Geometry check sheet. Reference: the model listing, model coordinates, mm. A direction names the side the tool comes from. Coordinates: 2 decimals unless noted, no trailing zeros. Write each loop counter-clockwise with the first axis right and the second up, starting at its lowest first coordinate (ties: lowest second). Pieces come first, ordered by that corner, then holes. Notation, with made-up numbers: (43.5, 63.5) -> (55.5, 63.5) arc R21 ccw to (55.5, 89.5) -> close; hole circle Ø4 at (-13.75, -30). An arc over 180 degrees is marked (long way). Answer in a Markdown table with one row per item. Add a question column.
1. Set-up check for faces 1 (the flat face through (12, 30, -48)), 2 (the flat face through (0, 9, 9)), 3 (the cylindrical face through (13.5, 4.4, 3.9)), 4 (the flat face through (0, 47, -52)), 5 (the flat face through (-4, 43, -30)): record each of +Z, -Z, +X, -X, +Y, -Y from which the full face is reachable in a straight line by a thin tool's end or side.
2. Scan lines: L1, parallel to Z at x = -10, y = 32; L2, parallel to Y at x = -5.75, z = -40; L3, parallel to Z at x = 18, y = 36. Record each from-to range of solid material in increasing order. Write a range as from..to.
3. Depth check by flat-ended pin: P1, Ø19, axis at y = 38.5, z = -33.5, coming from the +X side; P2, Ø5, axis at x = -7.5, y = 29, coming from the +Z side; P3, Ø6.5, axis at x = -16, y = 40, coming from the -Z side. Enter the tip coordinate at first touch or a pass-through.
4. Mould release check, pull along Z, two halves, no side actions. Record for faces 6 (the flat face through (0, 44, -8)), 7 (the cylindrical face through (0.056, 65.632, -54.374)), 8 (the cylindrical face through (17.352, 73.563, -35.708)), 9 (the cylindrical face through (-14.648, 73.563, -35.708)): pulls with the +Z half, pulls with the -Z half, needs draft (parallel to the pull), parting line crosses it, or undercut.
5. Cross-section at D-D on y = 72. Record the cut outline in (x, z), and give its area (3 significant figures).
6. Cross-section at C-C on y = 52. Record the cut outline in (x, z).
7. Cross-section at B-B on z = 1.5. Record the cut outline in (x, y).
8. Cross-section at A-A on x = -5. Record the cut outline in (y, z), and give its area (3 significant figures).
```python
from build123d import *
from build123d.topology import SkipClean

# Parameters (mm, degrees)
BASE_FOOT_WITH_SLOT_DEPTH     = 9
UPRIGHT_WALL_SKETCH_W         = 50
UPRIGHT_WALL_SKETCH_H         = 69
UPRIGHT_WALL_DEPTH            = 12
TOP_FLANGE_SKETCH_R           = 4.5
TOP_FLANGE_WITH_2_HOLES_DEPTH = 9
SIDE_BOSS_SKETCH_R            = 12
SIDE_BOSS_SKETCH_R_2          = 8
SIDE_BOSS_DEPTH               = 12
BOSS_WEB_DEPTH                = 4
BOSS_BORE_SKETCH_R            = 8
BOSS_BORE_DEPTH               = 102.434708064


with BuildPart() as part:
    # Base Foot Sketch → Base Foot with Slot (new body)
    with BuildSketch(Plane(origin=(0, 0, 0), x_dir=(1, 0, 0), z_dir=(0, 1, 0))):
        with BuildLine():
            Line((-25, 20), (25, 20))
            Line((25, 20), (25, -4))
            ThreePointArc((25, -4), (20.313708499, -15.313708499), (9, -20))
            Line((9, -20), (-9, -20))
            ThreePointArc((-9, -20), (-20.313708499, -15.313708499), (-25, -4))
            Line((-25, -4), (-25, 20))
        make_face()
        with BuildLine():
            Line((-9, 0.5), (9, 0.5))
            ThreePointArc((9, 0.5), (13.5, -4), (9, -8.5))
            Line((9, -8.5), (-9, -8.5))
            ThreePointArc((-9, -8.5), (-13.5, -4), (-9, 0.5))
        make_face(mode=Mode.SUBTRACT)
    extrude(amount=BASE_FOOT_WITH_SLOT_DEPTH)

    # Upright Wall Sketch → Upright Wall (add)
    with BuildSketch(Plane(origin=(0, 0, -20), x_dir=(-1, 0, 0), z_dir=(0, 0, -1))):
        with Locations((0, 43.5)):
            Rectangle(UPRIGHT_WALL_SKETCH_W, UPRIGHT_WALL_SKETCH_H)
    extrude(amount=-UPRIGHT_WALL_DEPTH)

    # Top Flange Sketch → Top Flange with 2 Holes (add)
    with BuildSketch(Plane(origin=(0, 78, 0), x_dir=(1, 0, 0), z_dir=(0, 1, 0))):
        with BuildLine():
            Line((-25, 20), (-25, 49))
            ThreePointArc((-25, 49), (-22.363961031, 55.363961031), (-16, 58))
            Line((-16, 58), (16, 58))
            ThreePointArc((16, 58), (22.363961031, 55.363961031), (25, 49))
            Line((25, 49), (25, 20))
            Line((25, 20), (-25, 20))
        make_face()
        with Locations(Location((-16, 40, 0), (0, 0, 270))):
            Circle(TOP_FLANGE_SKETCH_R, mode=Mode.SUBTRACT)
        with Locations(Location((16, 40, 0), (0, 0, 270))):
            Circle(TOP_FLANGE_SKETCH_R, mode=Mode.SUBTRACT)
    extrude(amount=-TOP_FLANGE_WITH_2_HOLES_DEPTH)



with BuildPart() as body_2:
    # Side Boss Sketch → Side Boss (new, symmetric)
    with BuildSketch(Plane(origin=(0, 0, 0), x_dir=(0, 0, -1), z_dir=(1, 0, 0))):
        with Locations((40, 32)):
            Circle(SIDE_BOSS_SKETCH_R)
        with Locations((40, 32)):
            Circle(SIDE_BOSS_SKETCH_R_2, mode=Mode.SUBTRACT)
    extrude(amount=SIDE_BOSS_DEPTH, both=True)


with BuildPart() as part_1:
    with SkipClean():  # the faces are left unmerged after this step: merging them gives an invalid solid
        add(part.part)

        add(body_2.part)  # Boss Web merges body 2
        # Boss Web Sketch → Boss Web (add, symmetric)
        with BuildSketch(Plane(origin=(0, 0, 0), x_dir=(0, 0, -1), z_dir=(1, 0, 0))):
            with BuildLine():
                Line((52, 32), (52, 61.444590884))
                ThreePointArc((52, 61.444590884), (54.416944157, 65.68531935), (58, 69))
                Line((58, 69), (20, 69))
                Line((20, 69), (20, 0))
                Line((20, 0), (46.285769513, 21.778008921))
                ThreePointArc((46.285769513, 21.778008921), (50.474474549, 26.144627858), (52, 32))
            make_face()
        extrude(amount=BOSS_WEB_DEPTH, both=True)

    # Boss Bore Sketch → Boss Bore (cut, through all)
    with SkipClean():  # the faces are left unmerged after this step: merging them gives an invalid solid
        with BuildSketch(Plane.ZY.offset(4)):
            with Locations(Location((-40, 32, 0), (0, 0, 180))):
                Circle(BOSS_BORE_SKETCH_R)
        extrude(amount=-BOSS_BORE_DEPTH, mode=Mode.SUBTRACT)


solid = part_1.part
```
Results found:
| question | item | result |
|---|---|---|
| 1 | face 1 | -Z, +X, -Y |
| 1 | face 2 | +Z, +X, -X, +Y |
| 1 | face 3 | +Y, -Y |
| 1 | face 4 | -Z, +X, -X, -Y |
| 1 | face 5 | -X |
| 2 | L1 | z = -52..-48, -32..-28, -20..-8 |
| 2 | L2 | y = 20..24, 40..44, 69..78 |
| 2 | L3 | z = -20..-8 |
| 3 | P1 | stops at x = 12 |
| 3 | P2 | stops at z = -8 |
| 3 | P3 | stops at z = -20 |
| 4 | face 6 | pulls with the +Z half |
| 4 | face 7 | pulls with the -Z half |
| 4 | face 8 | undercut |
| 4 | face 9 | undercut |
| 5 | outline | (-25, -49) arc R9 ccw to (-16, -58) -> (16, -58) arc R9 ccw to (25, -49) -> (25, -8) -> (-25, -8) -> close; hole circle Ø9 at (-16, -40); hole circle Ø9 at (16, -40) |
| 5 | area | 2,340 mm^2 |
| 6 | outline | (-25, -20) -> (-4, -20) -> (-4, -52) -> (4, -52) -> (4, -20) -> (25, -20) -> (25, -8) -> (-25, -8) -> close |
| 7 | outline | (-25, 0) -> (-12.74, 0) -> (-12.74, 9) -> (-25, 9) -> close; (12.74, 0) -> (25, 0) -> (25, 9) -> (12.74, 9) -> close |
| 8 | outline | (0, -20) -> (69, -20) -> (69, -58) -> (78, -58) -> (78, -8) -> (9, -8) -> (9, -0.5) -> (0, -0.5) -> close; (0, 8.5) -> (9, 8.5) -> (9, 20) -> (0, 20) -> close; circle Ø24 at (32, -40); hole circle Ø16 at (32, -40) |
| 8 | area | 1,700 mm^2 |
